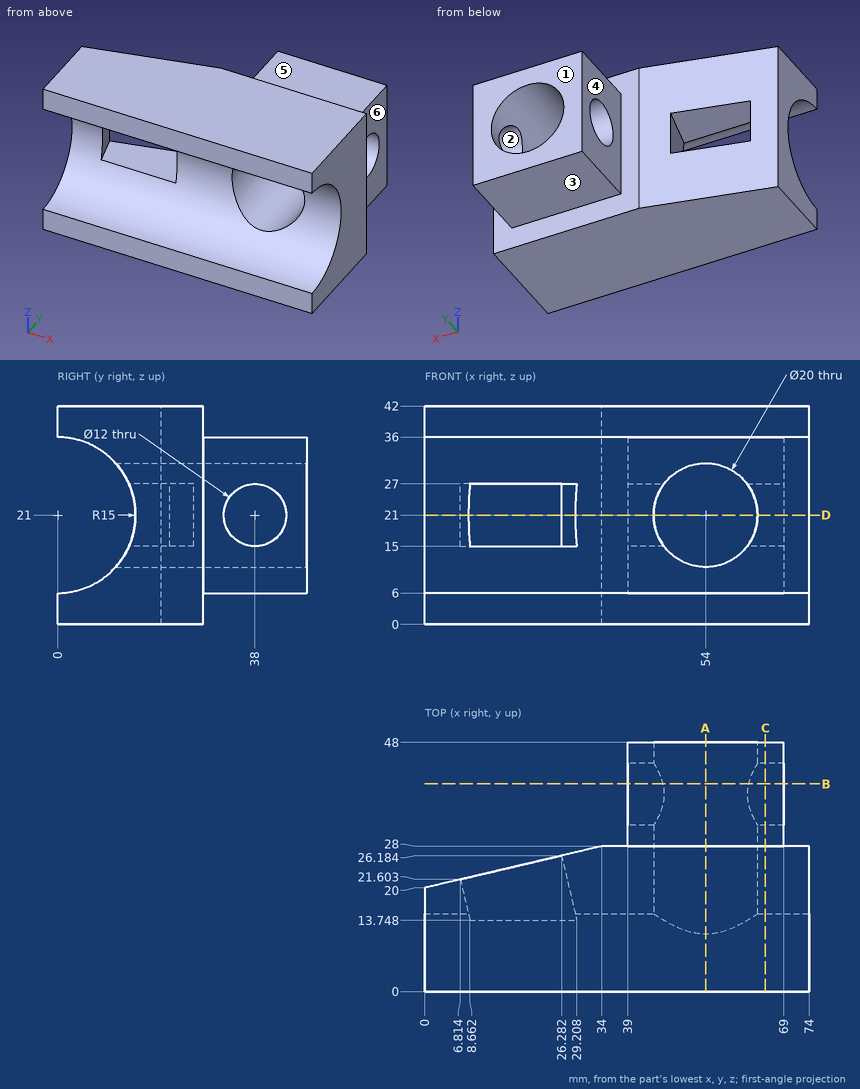
Study the drawing (mm; zero at the part's minimum x, y, z) and answer. A direction names the side the tool comes from. Coordinates: 2 decimals unless noted, no trailing zeros. Loops run counter-clockwise (first coordinate to the right, second up) from the corner with the lowest first, then second, coordinate; pieces in that order, holes last. Notation, with made-up numbers: M -21,44.5 L 0,44.5 A30 ccw 0,79.5 Z; hole C 31,34.5 d7. An arc over 180 degrees is marked long. Answer as a JSON object with one key per item and string values. Group by question number.
Item 1: Consider L1, parallel to Y at x = 43, z = 21; L2, parallel to Y at x = 68.5, z = 23 (1 decimal); L3, parallel to X at y = 23, z = 21. Determine where each line is inside the solid, lowest interval first.
Item 2: Section B-B (y = 40) is taken. Write down the section's boundary in (x, z).
Item 3: Which of the six approach directions +Z, -Z, +X, -X, +Y, -Y give full straight-line access (tool end or side, diameter ignored) to the marked faces 4, 5 and 6?
Item 4: Section D-D (z = 21) is taken. Write down the section's boundary in (x, y).
Item 5: Each of these flat-tipped pins is pushed along its axis until it touches: P1, Ø16, axis at x = 53.5, y = 42.5, coming from the -Z side; P2, Ø14, axis at y = 38, z = 21, coming from the -X side; P3, Ø5, axis at x = 22.5, z = 5, coming from the +Y side; P4, Ø6, axis at y = 35.5, z = 22, coming from the +X side. Where does it stop, or does it pass through?
Item 6: Section C-C (x = 65.5) is taken. Write down the section's boundary in (y, z), and give its area (3 significant figures).
Item 7: Section A-A (x = 54) is taken. Write down the section's boundary in (y, z).
Item 8: Determine the mould class of the marked faces 1, 2 and 3 for opening direction Y: +Y half, -Y half, draft (parallel to the pull), parting line (faces both ways), or undercut.
Solved:
{
 "1": {"L1": "y = 15 to 32, 44 to 48", "L2": "y = 14.9 to 32.3, 43.7 to 48", "L3": "x = 27.03 to 44, 64 to 74"},
 "2": {"outline": "M 39,6 L 69,6 L 69,15.34 L 62.25,15.34 A10 cw 45.75,15.34 L 39,15.34 Z; M 39,26.66 L 45.75,26.66 A10 cw 62.25,26.66 L 69,26.66 L 69,36 L 39,36 Z"},
 "3": {"face 4": "+Z, -Z, -X, +Y", "face 5": "+Z, +X, -X, +Y", "face 6": "+Z, -Z, +X, +Y"},
 "4": {"outline": "M 0,15 L 8.37,15 L 6.81,21.6 L 0,20 Z; M 26.28,26.18 L 28.91,15 L 44,15 L 44,32 L 39,32 L 39,28 L 34,28 Z; M 39,44 L 44,44 L 44,48 L 39,48 Z; M 64,15 L 74,15 L 74,28 L 69,28 L 69,32 L 64,32 Z; M 64,44 L 69,44 L 69,48 L 64,48 Z"},
 "5": {"P1": "stops at z = 6", "P2": "stops at x = 39", "P3": "stops at y = 25.88", "P4": "passes through"},
 "6": {"outline": "M 0,0 L 28,0 L 28,6 L 48,6 L 48,36 L 28,36 L 28,42 L 0,42 L 0,36 A15 cw 0,6 Z; hole C 38,21 d12", "area": "1,310 mm2"},
 "7": {"outline": "M 0,0 L 28,0 L 28,6 L 48,6 L 48,11 L 11.18,11 A15 cw 0,6 Z; M 0,36 A15 cw 11.18,31 L 48,31 L 48,36 L 28,36 L 28,42 L 0,42 Z"},
 "8": {"face 1": "+Y half", "face 2": "undercut", "face 3": "draft"}
}
